```python
from build123d import *

# Parameters (mm, degrees)
SKETCH_1_R               = 160
SKETCH_1_R_2             = 125
EXTRUDE_1_DEPTH          = 4
SKETCH_2_R               = 3
CUT_EXTRUDE_1_DEPTH      = 227.309522557
PATTERN_CIRCULAR_1_COUNT = 8


with BuildPart() as part:
    # 草图1 → 凸台-拉伸1 (new body)
    with BuildSketch(Plane(origin=(0, 0, 0), x_dir=(1, 0, 0), z_dir=(0, 1, 0))):
        with Locations(Location((0, 0, 0), (0, 0, 270))):
            Circle(SKETCH_1_R)
        with Locations(Location((0, 0, 0), (0, 0, 270))):
            Circle(SKETCH_1_R_2, mode=Mode.SUBTRACT)
    extrude(amount=EXTRUDE_1_DEPTH)

    # 草图2 → 切除-拉伸1 (cut, through all)
    with BuildSketch(Plane(origin=(0, 4, 0), x_dir=(1, 0, 0), z_dir=(0, 1, 0))):
        with Locations(Location((0, 145, 0), (0, 0, 270))):
            Circle(SKETCH_2_R)
    cut_extrude_1 = extrude(amount=-CUT_EXTRUDE_1_DEPTH, mode=Mode.SUBTRACT)

    # 阵列(圆周)1: 切除-拉伸1 ×8 about axis
    pattern_circular_1_axis = Axis((0, 0, 0), (0, 1, 0))
    for i in range(1, PATTERN_CIRCULAR_1_COUNT):
        add(cut_extrude_1.rotate(pattern_circular_1_axis, i * 360 / PATTERN_CIRCULAR_1_COUNT), mode=Mode.SUBTRACT)


solid = part.part
```
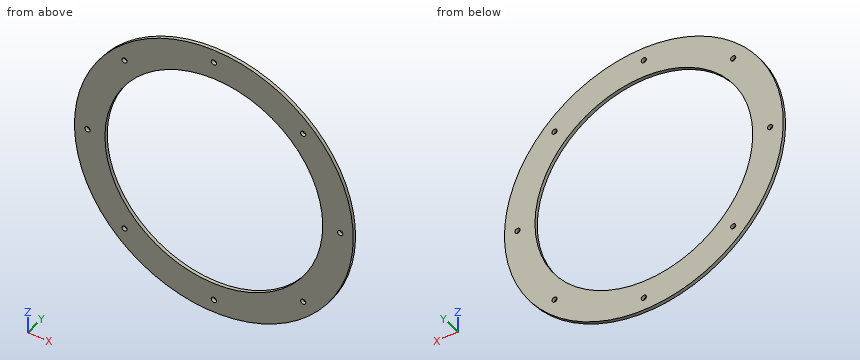
Geometry check sheet. Reference: the model listing, model coordinates, mm. Give positions to 0.01 mm unless a question says otherwise; leave off trailing zeros. Loops run counter-clockwise (first coordinate to the right, second up) from the corner with the lowest first, then second, coordinate; pieces in that order, holes last. Notation, with made-up numbers: M -34.5,63.25 L -20.5,63.25 A18 ccw -20.5,96.25 Z; hole C 0,-5 d11. An arc over 180 degrees is marked long. Write item = value, one per line.
(1) Material ranges on line 1 (X direction, y = 2.85, z = 147.5); line 2 (X direction, y = 0.95, z = -58); line 3 (Z direction, x = -111, y = 1.05), recorded low to high. Write a range as [from, to].
Answer below:
line_1 = [-62, -1.66], [1.66, 62]
line_2 = [-149.12, -110.73], [110.73, 149.12]
line_3 = [-115.23, -57.48], [57.48, 115.23]
(2) Sectioned sample at C-C, the plane y = 0.7. State how many separate pieces and enclosed holes the cut face has, plus the area to 3 significant figures.
Answer below:
separate_pieces = 1
enclosed_holes = 9
area = 31,100 mm2
(3) Gauge pin test, flat ends, axial feed: pin 1 Ø1 at (x, y) = (22.5, 3) entering from +Z; pin 2 Ø1.5 at (y, z) = (3.5, 101) entering from +X; pin 3 Ø1.5 at (x, y) = (125, 1.5) entering from +Z. Record the tip position at first contact, or that the pin passes through.
Answer below:
pin_1 = 158.48
pin_2 = 124.7
pin_3 = 100.81
(4) Sectioned sample at B-B, the plane x = 44.5. Record the cut outline in (y, z), plus the area to 3 significant figures.
Answer below:
outline = M 0,-153.69 L 4,-153.69 L 4,-116.81 L 0,-116.81 Z; M 0,116.81 L 4,116.81 L 4,153.69 L 0,153.69 Z
area = 295 mm2
(5) Sectioned sample at A-A, the plane z = 50. Record the cut outline in (x, y), plus the area to 3 significant figures.
Answer below:
outline = M -151.99,0 L -114.56,0 L -114.56,4 L -151.99,4 Z; M 114.56,0 L 151.99,0 L 151.99,4 L 114.56,4 Z
area = 299 mm2
(6) Sectioned sample at D-D, the plane z = 132.5. Record the cut outline in (x, y).
Answer below:
outline = M -89.69,0 L 89.69,0 L 89.69,4 L -89.69,4 Z
